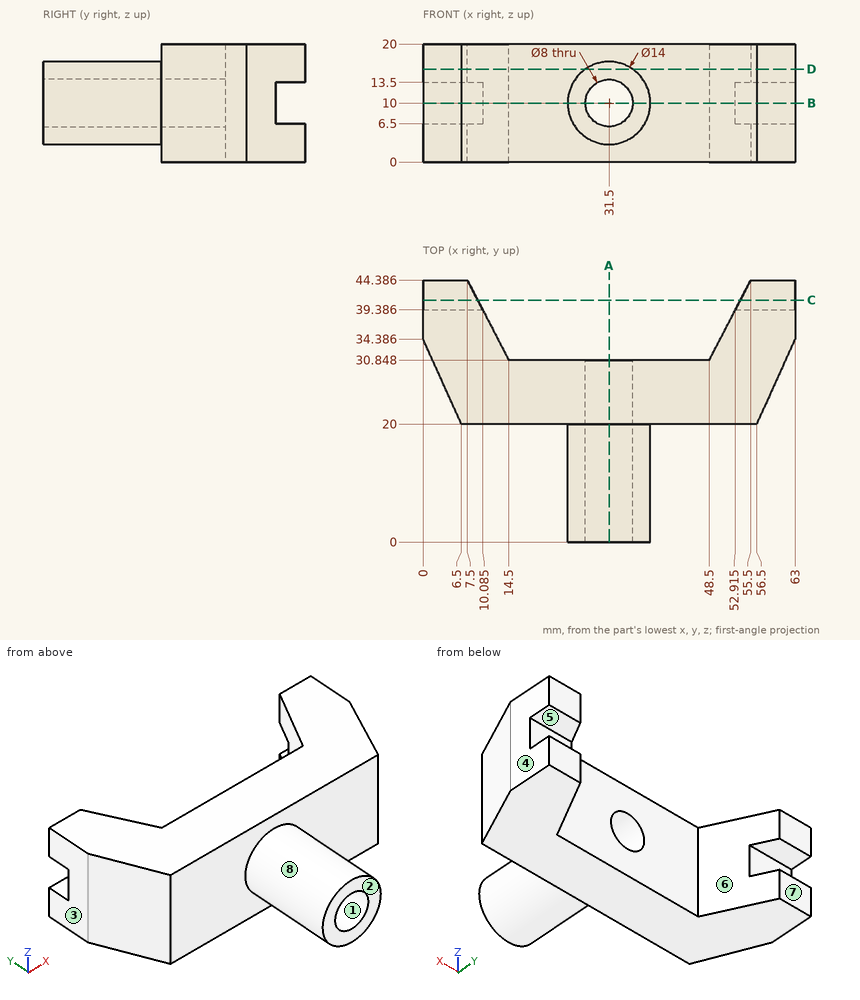
Verification items for this drawing (mm, ordinates from the low corner). A direction names the side the tool comes from. Give positions to 0.01 mm unless a question says otherwise; leave off trailing zeros. Order: outer loops, then holes, each group sorted by start corner. A loop starts at its lowest first (then second) coordinate and runs counter-clockwise, first axis right, second up. Notation, with made-up numbers: M -15.75,-11 L 25.25,-11 A34 cw 25.25,22 Z; hole C 86,-17.75 d3. An arc over 180 degrees is marked long. Use a Markdown table: item, result.
Item 1: Section check B-B (z = 10). Record the cut outline in (x, y) (1 decimal).
Answers follow:
| item | result |
|---|---|
| outline | M 0,34.4 L 6.5,20 L 24.5,20 L 24.5,0 L 27.5,0 L 27.5,30.8 L 14.5,30.8 L 10.1,39.4 L 0,39.4 Z; M 35.5,0 L 38.5,0 L 38.5,20 L 56.5,20 L 63,34.4 L 63,39.4 L 52.9,39.4 L 48.5,30.8 L 35.5,30.8 Z |
Item 2: Section check C-C (y = 41). Record the cut outline in (x, z).
Answers follow:
| item | result |
|---|---|
| outline | M 0,0 L 9.25,0 L 9.25,6.5 L 0,6.5 Z; M 0,13.5 L 9.25,13.5 L 9.25,20 L 0,20 Z; M 53.75,0 L 63,0 L 63,6.5 L 53.75,6.5 Z; M 53.75,13.5 L 63,13.5 L 63,20 L 53.75,20 Z |
Item 3: Depth check by flat-ended pin: P1, Ø5.5, axis at x = 3, z = 10, coming from the +Y side; P2, Ø1.5, axis at x = 55.5, y = 41, coming from the -Z side; P3, Ø1.5, axis at x = 26.5, z = 5.5, coming from the +Y side; P4, Ø2, axis at y = 17.5, z = 10, coming from the -X side. Enter the tip coordinate at first touch or a pass-through.
Answers follow:
| item | result |
|---|---|
| P1 | stops at y = 39.39 |
| P2 | stops at z = 0 |
| P3 | stops at y = 30.85 |
| P4 | stops at x = 24.5 |
Item 4: Draft check along X on the marked faces 1, 2 and 3. Enter one of: +X half, -X half, draft (parallel to the pull), parting line (faces both ways), or undercut.
Answers follow:
| item | result |
|---|---|
| face 1 | undercut |
| face 2 | draft |
| face 3 | -X half |
Item 5: Section check D-D (z = 15.75). Record the cut outline in (x, y) (1 decimal).
Answers follow:
| item | result |
|---|---|
| outline | M 0,34.4 L 6.5,20 L 27.5,20 L 27.5,0 L 35.5,0 L 35.5,20 L 56.5,20 L 63,34.4 L 63,44.4 L 55.5,44.4 L 48.5,30.8 L 14.5,30.8 L 7.5,44.4 L 0,44.4 Z |
Item 6: Tool access check on the marked faces 4, 5, 6, 7 and 8. Record the directions out of +Z, -Z, +X, -X, +Y, -Y that give a thin tool (end or side, any length) a straight path to the whole face; none if there is none.
Answers follow:
| item | result |
|---|---|
| face 4 | +Z, -Z, +X, +Y, -Y |
| face 5 | +X, -X, +Y |
| face 6 | +Z, -Z, +Y |
| face 7 | +Z, -Z, +X, -X, +Y |
| face 8 | -Y |
Item 7: Material ranges on line 1 along X through (y, z) = (4, 10); line 2 along Y through (x, z) = (38, 8.5); line 3 along Y through (x, z) = (21.5, 19), recorded low to high.
Answers follow:
| item | result |
|---|---|
| line 1 | x = 24.5 to 27.5, 35.5 to 38.5 |
| line 2 | y = 0 to 30.85 |
| line 3 | y = 20 to 30.85 |
Item 8: Section check A-A (x = 31.5). Record the cut outline in (y, z), and give its area (3 significant figures).
Answers follow:
| item | result |
|---|---|
| outline | M 0,3 L 20,3 L 20,0 L 30.85,0 L 30.85,6 L 0,6 Z; M 0,14 L 30.85,14 L 30.85,20 L 20,20 L 20,17 L 0,17 Z |
| area | 250 mm2 |
